from build123d import *

# Parameters (mm, degrees)
CROSSRECESS_DEPTH = 1.65
DRAFT9_ANGLE      = 30
FILLET5_R         = 0.3
SKETCH10_W        = 1
SKETCH10_H        = 3


with BuildPart() as part:
    # Sketch1 → Base (revolve)
    with BuildSketch(Plane.XY, mode=Mode.PRIVATE) as base_sk:
        Polygon((75, 3), (5.3, 3), (3.3, 3), (0.85, 5.45), (0, 5.45), (0, 0), (75, 0), align=None)
    revolve(base_sk.sketch.rotate(Axis((4.515812911, 0, 0), (-1, 0, 0)), 90), axis=Axis((4.515812911, 0, 0), (-1, 0, 0)))

    # Sketch6 → CrossRecess (cut)
    with BuildSketch(Plane(origin=(0, 0, 0), x_dir=(0, 0, -1), z_dir=(1, 0, 0))):
        Polygon((0.68, 0.68), (0.68, 3.4), (-0.68, 3.4), (-0.68, 0.68), (-3.4, 0.68), (-3.4, -0.68), (-0.68, -0.68), (-0.68, -3.4), (0.68, -3.4), (0.68, -0.68), (3.4, -0.68), (3.4, 0.68), align=None)
    extrude(amount=CROSSRECESS_DEPTH, mode=Mode.SUBTRACT)

    # Draft9
    draft9_faces = [part.faces().sort_by_distance(p)[0] for p in [
        (0.825, -3.4, 0),
        (0.825, 0, 3.4),
        (0.825, 0, -3.4),
        (0.825, 3.4, 0),
    ]]
    draft(draft9_faces, Plane(origin=(0, 5.45, 0), x_dir=(0, 0, -1), z_dir=(-1, 0, 0)), DRAFT9_ANGLE)

    # Fillet5
    fillet5_edges = [part.edges().sort_by_distance(p)[0] for p in [
        (0.825, 0.68, 0.68),
        (0.825, -0.68, 0.68),
        (0.825, -0.68, -0.68),
        (0.825, 0.68, -0.68),
    ]]
    fillet(fillet5_edges, radius=FILLET5_R)

    # Sketch10 → Revolve2 (revolve)
    with BuildSketch(Plane.XY):
        with Locations((3.8, 1.5)):
            Rectangle(SKETCH10_W, SKETCH10_H)
    revolve(axis=Axis((62.228915663, 0, 0), (-1, 0, 0)))


solid = part.part
Model file for the job. Use its own axes, mm. A direction names the side the tool comes from. Coordinates: 2 decimals unless noted, no trailing zeros. Order: outer loops, then holes, each group sorted by start corner. A loop starts at its lowest first (then second) coordinate and runs counter-clockwise, first axis right, second up. Notation, with made-up numbers: (-34, 83) -> (-1, 83) arc R22 ccw to (-1, 101) -> close; hole circle Ø7 at (35, -26). An arc over 180 degrees is marked (long way). Return JSON: item names as keys, results as strings. Group by question number.
Item 1: Pull direction Y, two halves, no side cores. Call faces 4 (the flat face through (75, 0, 0)), 5 (the flat face through (0.813, -0.01, -2.93)), 6 (the conical face through (3.147, -3.126, 0.41)): pulls with the +Y half, pulls with the -Y half, needs draft (parallel to the pull), parting line crosses it, or undercut.
Item 2: Saw through at A-A on y = 0. Write the cut outline in (x, z), then the cut area to 3 significant figures.
Item 3: Wall check: line 1 along X through (y, z) = (-0.5, 0.5); line 2 along Z through (x, y) = (45, -1.75); line 3 along Z through (x, y) = (60, 0.25). Give the ranges that are in metal, low to high. Write a range as [from, to].
Item 4: Flat gauge pins, fed straight in: P1, Ø1, axis at x = 45, z = -1.5, coming from the -Y side; P2, Ø0.8, axis at x = 0.5, z = -2, coming from the +Y side; P3, Ø1.3, axis at x = 0.5, y = 2, coming from the +Z side; P4, Ø4, axis at y = 0.5, z = 1, coming from the -X side. Where does each tip first touch, or does it go through?
Item 5: Saw through at C-C on x = 57. Write the cut outline in (y, z), then the cut area to 3 significant figures.
Item 6: Tool access for faces 1 (the cylindrical face through (0.419, 4.835, -2.515)), 2 (the cylindrical face through (38.65, -0.9, -2.86)), 3 (the flat face through (0.813, 2.93, -0.01)): list every direction of +Z, -Z, +X, -X, +Y, -Y with a clear straight run to the whole face (end or side of a thin tool).
Values found:
{
 "1": {"face 4": "needs draft", "face 5": "undercut", "face 6": "parting line crosses it"},
 "2": {"outline": "(0, -5.45) -> (0.85, -5.45) -> (3.3, -3) -> (75, -3) -> (75, 3) -> (3.3, 3) -> (0.85, 5.45) -> (0, 5.45) -> (0, 3.4) -> (1.65, 2.45) -> (1.65, -2.45) -> (0, -3.4) -> close", "area": "451 mm2"},
 "3": {"line 1": "x = [1.65, 75]", "line 2": "z = [-2.44, 2.44]", "line 3": "z = [-2.99, 2.99]"},
 "4": {"P1": "stops at y = -2.83", "P2": "stops at y = 5.21", "P3": "stops at z = 5.28", "P4": "stops at x = 0"},
 "5": {"outline": "circle Ø6 at (0, 0)", "area": "28.3 mm2"},
 "6": {"face 1": "+X, -X", "face 2": "+X", "face 3": "-X"}
}
